Here's how the part is built. I have some questions about the finished solid (model axes, mm). A direction names the side the tool comes from. Coordinates: 2 decimals unless noted, no trailing zeros. Write each loop counter-clockwise with the first axis right and the second up, starting at its lowest first coordinate (ties: lowest second). Pieces come first, ordered by that corner, then holes.
Item 1: I'm going to push flat-ended pins straight in: pin 1 Ø2 at (y, z) = (0, -5) entering from -X; pin 2 Ø1 at (y, z) = (-0.5, 4) entering from -X; pin 3 Ø1.5 at (y, z) = (2.5, -1) entering from -X. Where does each tip first touch, or does it pass through?
Item 2: If we section it at C-C (y = 1.7): Please give me the cut outline in (x, z), then the cut area to 3 significant figures.
Item 3: We'd pull the mould along Z, two halves only. Please class faces 1 (the face through (-2, 0, 0)), 2 (the face through (0, -3, 3)), 3 (the face through (4.412, -0.125, -1.389)): +Z half, -Z half, draft (parallel to the pull), parting line (faces both ways), or undercut.
Item 4: If we section it at A-A (x = 0): Please give me the cut outline in (y, z), then the cut area to 3 significant figures.
Item 5: If we section it at B-B (y = -0.95): Please give me the cut outline in (x, z).
Item 6: For faces 4 (the face through (4.412, 0.125, -1.389)), 5 (the face through (0, 3, 3)), which set-ups out of +Z, -Z, +X, -X, +Y, -Y let a thin tool reach every point of the face, with its end or its side?
Item 7: If I drill on line 1 (Y direction, x = -6, z = 0.25); line 2 (Z direction, x = 0.75, y = -2.7); line 3 (Z direction, x = -1.75, y = -0.85), over which ranges is the centre line in solid material (lowest first)?
from build123d import *

# Parameters (mm, degrees)
SKETCH_1_R          = 4.5
SKETCH_2_R          = 6.5
SKETCH_3_R          = 6.5
EXTRUDE_1_DEPTH     = 1
SKETCH_4_R          = 2
CUT_EXTRUDE_1_DEPTH = 11.977249318
CHAMFER_1_SIZE      = 0.2


with BuildPart() as part:
    # 草图1 → 放样1 section 0
    with BuildSketch(Plane(origin=(0, 0, 0), x_dir=(1, 0, 0), z_dir=(0, 1, 0))):
        Circle(SKETCH_1_R)
    # 草图2 → 放样1 section 1
    with BuildSketch(Plane(origin=(0, 2, 0), x_dir=(1, 0, 0), z_dir=(0, 1, 0))):
        Circle(SKETCH_2_R)
    loft_1 = loft()

    # 草图3 → 凸台-拉伸1 (add)
    with BuildSketch(Plane(origin=(0, 2, 0), x_dir=(1, 0, 0), z_dir=(0, 1, 0))):
        with Locations(Location((0, 0, 0), (0, 0, 270))):
            Circle(SKETCH_3_R)
    extrude_1 = extrude(amount=EXTRUDE_1_DEPTH)

    # 镜向1: 放样1, 凸台-拉伸1 across plane
    add(loft_1.mirror(Plane.ZX))
    add(extrude_1.mirror(Plane.ZX))

    # 草图4 → 切除-拉伸1 (cut, through all)
    with BuildSketch(Plane(origin=(0, 3, 0), x_dir=(1, 0, 0), z_dir=(0, 1, 0))):
        with Locations(Location((0, 0, 0), (0, 0, 270))):
            Circle(SKETCH_4_R)
    extrude(amount=-CUT_EXTRUDE_1_DEPTH, mode=Mode.SUBTRACT)

    # 倒角1
    chamfer_1_edges = [part.edges().sort_by_distance(p)[0] for p in [
        (0, -3, -2),
        (0, 3, -2),
    ]]
    chamfer(chamfer_1_edges, length=CHAMFER_1_SIZE)


solid = part.part
Answer list:
1. pin 1: stops at x = -2.96
1. pin 2: stops at x = -3.93
1. pin 3: stops at x = -6.5
2. outline: circle Ø12.4 at (0, 0); hole circle Ø4 at (0, 0)
2. area: 108 mm2
3. face 1: undercut
3. face 2: draft
3. face 3: parting line
4. outline: (-3, -6.5) - (-2, -6.5) - (0, -4.5) - (2, -6.5) - (3, -6.5) - (3, -2.2) - (2.8, -2) - (-2.8, -2) - (-3, -2.2) - close; (-3, 2.2) - (-2.8, 2) - (2.8, 2) - (3, 2.2) - (3, 6.5) - (2, 6.5) - (0, 4.5) - (-2, 6.5) - (-3, 6.5) - close
4. area: 45.9 mm2
5. outline: circle Ø10.9 at (0, 0); hole circle Ø4 at (0, 0)
6. face 4: none
6. face 5: +Z, -Z, +X, -X, +Y
7. line 1: y = -3 to -1.51, 1.51 to 3
7. line 2: z = -6.46 to -1.85, 1.85 to 6.46
7. line 3: z = -5.06 to -0.97, 0.97 to 5.06
